Can you work these out from the model? Positions are in its coordinate system, mm. Face numbers are marked on the shaded views. Give positions to 0.01 mm unless a question says otherwise; leave off trailing zeros. Write each loop counter-clockwise with the first axis right and the second up, starting at its lowest first coordinate (ties: lowest second). Pieces come first, ordered by that corner, then holes. Notation, with made-up numbers: (-23.5, 41.5) -> (-15.5, 41.5) arc R15 ccw to (-15.5, 56.5) -> close; hole circle Ø6 at (19.5, 63). An arc over 180 degrees is marked (long way). One line per item, written item: value.
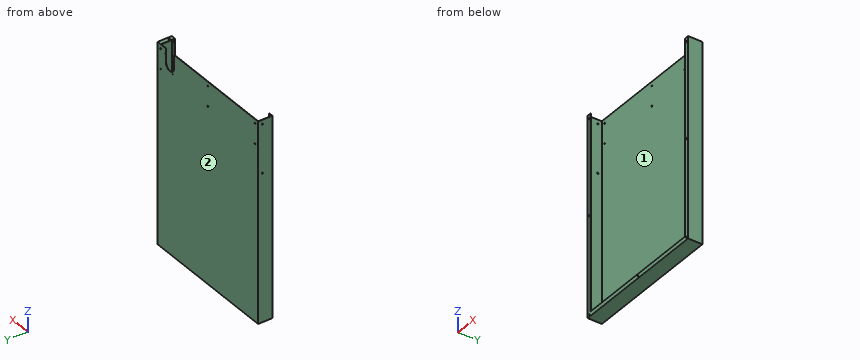
from build123d import *

# Parameters (mm, degrees)
SKETCH_1_W             = 980
SKETCH_1_H             = 1400
EXTRUDE_1_DEPTH        = 100
SHELL_1_T              = -2
CUT_EXTRUDE_1_DEPTH    = 20
SKETCH_5_W             = 976
SKETCH_5_H             = 98
CUT_EXTRUDE_2_DEPTH    = 20
EXTRUDE_2_DEPTH        = 2
SKETCH_7_W             = 2
SKETCH_7_H             = 96
EXTRUDE_3_DEPTH        = 28
SKETCH_8_R             = 4.5
CUT_EXTRUDE_3_DEPTH    = 10
SKETCH_9_R             = 4.5
CUT_EXTRUDE_4_DEPTH    = 10
SKETCH_10_R            = 4.5
CUT_EXTRUDE_5_DEPTH    = 10
SKETCH_11_R            = 4.5
CUT_EXTRUDE_6_DEPTH    = 10
HOLE_WIZARD_M5_1_D     = 4.2
HOLE_WIZARD_M5_1_DEPTH = 1260
HOLE_WIZARD_M5_1_TIP   = 1.2618073


with BuildPart() as part:
    # 草图1 → 凸台-拉伸1 (new body)
    with BuildSketch(Plane(origin=(0, 0, 0), x_dir=(1, 0, 0), z_dir=(0, 1, 0))):
        Rectangle(SKETCH_1_W, SKETCH_1_H)
    extrude(amount=-EXTRUDE_1_DEPTH)

    # 抽壳1
    shell_1_openings = [part.faces().sort_by_distance(p)[0] for p in [
        (0, -100, 0),
    ]]
    offset(amount=SHELL_1_T, openings=shell_1_openings, kind=Kind.INTERSECTION)

    # 草图3 → 切除-拉伸1 (cut)
    with BuildSketch(Plane(origin=(0, 0, 0), x_dir=(1, 0, 0), z_dir=(0, 1, 0))):
        with BuildLine():
            Line((330, -700), (410, -700))
            Line((410, -700), (410, -604.5))
            ThreePointArc((410, -604.5), (370, -564.996875122), (330, -604.5))
            Line((330, -604.5), (330, -700))
        make_face()
    extrude(amount=-CUT_EXTRUDE_1_DEPTH, mode=Mode.SUBTRACT)

    # 草图5 → 切除-拉伸2 (cut)
    with BuildSketch(Plane.XY.offset(700)):
        with Locations((0, -51)):
            Rectangle(SKETCH_5_W, SKETCH_5_H)
    extrude(amount=-CUT_EXTRUDE_2_DEPTH, mode=Mode.SUBTRACT)

    # 草图6 → 凸台-拉伸2 (add)
    with BuildSketch(Plane.XZ.offset(100)):
        Polygon((490, 700), (490, -700), (-490, -700), (-490, 700), (-460, 700), (-460, -670), (460, -670), (460, 700), align=None)
    extrude(amount=-EXTRUDE_2_DEPTH)

    # 草图7 → 凸台-拉伸3 (add)
    with BuildSketch(Plane.ZY.offset(-488)):
        with Locations((699, -50)):
            Rectangle(SKETCH_7_W, SKETCH_7_H)
    extrude(amount=EXTRUDE_3_DEPTH)

    # 草图8 → 切除-拉伸3 (cut)
    with BuildSketch(Plane.XZ.offset(100)):
        with Locations(Location((-474, 670, 0), (0, 0, 270))):
            Circle(SKETCH_8_R)
        with Locations(Location((-474, 0, 0), (0, 0, 270))):
            Circle(SKETCH_8_R)
        with Locations(Location((-474, -684, 0), (0, 0, 270))):
            Circle(SKETCH_8_R)
        with Locations(Location((0, -684, 0), (0, 0, 270))):
            Circle(SKETCH_8_R)
        with Locations(Location((474, -684, 0), (0, 0, 270))):
            Circle(SKETCH_8_R)
        with Locations(Location((474, 0, 0), (0, 0, 270))):
            Circle(SKETCH_8_R)
        with Locations(Location((474, 670, 0), (0, 0, 270))):
            Circle(SKETCH_8_R)
    extrude(amount=-CUT_EXTRUDE_3_DEPTH, mode=Mode.SUBTRACT)

    # 草图9 → 切除-拉伸4 (cut)
    with BuildSketch(Plane(origin=(0, 0, 698), x_dir=(-1, 0, 0), z_dir=(0, 0, -1))):
        with Locations((-474, -70)):
            Circle(SKETCH_9_R)
    extrude(amount=-CUT_EXTRUDE_4_DEPTH, mode=Mode.SUBTRACT)

    # 草图10 → 切除-拉伸5 (cut)
    with BuildSketch(Plane(origin=(-488, 0, 0), x_dir=(0, 0, -1), z_dir=(1, 0, 0))):
        with Locations((-670, -30)):
            Circle(SKETCH_10_R)
        with Locations((-330, -30)):
            Circle(SKETCH_10_R)
    extrude(amount=-CUT_EXTRUDE_5_DEPTH, mode=Mode.SUBTRACT)

    # 草图11 → 切除-拉伸6 (cut)
    with BuildSketch(Plane(origin=(0, 0, 0), x_dir=(1, 0, 0), z_dir=(0, 1, 0))):
        with Locations(Location((-460, -670, 0), (0, 0, 270))):
            Circle(SKETCH_11_R)
        with Locations(Location((0, -530, 0), (0, 0, 270))):
            Circle(SKETCH_11_R)
        with Locations(Location((460, -530, 0), (0, 0, 270))):
            Circle(SKETCH_11_R)
        with Locations(Location((-460, -530, 0), (0, 0, 270))):
            Circle(SKETCH_11_R)
        with Locations(Location((0, -670, 0), (0, 0, 270))):
            Circle(SKETCH_11_R)
        with Locations(Location((460, -670, 0), (0, 0, 270))):
            Circle(SKETCH_11_R)
    extrude(amount=-CUT_EXTRUDE_6_DEPTH, mode=Mode.SUBTRACT)

    # M5 螺纹孔1
    with Locations(Plane(origin=(0, 0, 0), x_dir=(-1, 0, 0), z_dir=(0, 1, 0))):
        with Locations((-343, 558.234628196), (-316, 605), (-415, 659)):
            Hole(HOLE_WIZARD_M5_1_D / 2, depth=HOLE_WIZARD_M5_1_DEPTH)
            with Locations((0, 0, -(HOLE_WIZARD_M5_1_DEPTH + HOLE_WIZARD_M5_1_TIP / 2))):  # 118° drill point
                Cone(0, HOLE_WIZARD_M5_1_D / 2, HOLE_WIZARD_M5_1_TIP, mode=Mode.SUBTRACT)


solid = part.part
1) I need wall thicknesses on L1, parallel to Z at x = 474, y = -99; L2, parallel to X at y = -1, z = 605; L3, parallel to X at y = -99.3, z = 0. Which ranges of each line are inside material? Lowest first, please.
Answer list:
L1: z = -700 to -688.5, -679.5 to -4.5, 4.5 to 665.5, 674.5 to 700
L2: x = -490 to 313.9, 318.1 to 330, 410 to 490
L3: x = -490 to -478.5, -469.5 to -460, 460 to 469.5, 478.5 to 490
2) We'd pull the mould along X, two halves only. Please class the marked faces 1 and 2: released by +X, released by -X, zero draft, split by the parting line, or undercut.
Answer list:
face 1: undercut
face 2: zero draft
3) If we section it at C-C (x = -138.5): Write out the boundary of the cut face in (y, z), and give its area (3 significant figures).
Answer list:
outline: (-100, -700) -> (0, -700) -> (0, 700) -> (-2, 700) -> (-2, -698) -> (-98, -698) -> (-98, -670) -> (-100, -670) -> close
area: 3,050 mm^2
4) If we section it at B-B (z = 92.5): Write out the boundary of the cut face in (x, y), and give its area (3 significant figures).
Answer list:
outline: (-490, -100) -> (-460, -100) -> (-460, -98) -> (-488, -98) -> (-488, -2) -> (488, -2) -> (488, -98) -> (460, -98) -> (460, -100) -> (490, -100) -> (490, 0) -> (-490, 0) -> close
area: 2,460 mm^2
5) Will these pins go through, and if not, where does the flat tip stop? pin 1 (5.5 mm diameter, centred on x = 474, z = 0, fed in from -Y); pin 2 (1.6 mm diameter, centred on x = -39, y = -99, fed in from +Z); pin 3 (6 mm diameter, centred on x = -154, y = -81.5, fed in from +Z); pin 4 (3.5 mm diameter, centred on x = 316, z = 605, fed in from -Y).
Answer list:
pin 1: stops at y = -2
pin 2: stops at z = -670
pin 3: stops at z = -698
pin 4: passes through
6) If we section it at A-A (x = 370): Write out the boundary of the cut face in (y, z), and give its area (3 significant figures).
Answer list:
outline: (-100, -700) -> (0, -700) -> (0, 565) -> (-2, 565) -> (-2, -698) -> (-98, -698) -> (-98, -670) -> (-100, -670) -> close
area: 2,780 mm^2
